Part model, mm, in its own coordinate system. A direction names the side the tool comes from. Give positions to 0.01 mm unless a question says otherwise; leave off trailing zeros. Loops run counter-clockwise (first coordinate to the right, second up) from the corner with the lowest first, then second, coordinate; pieces in that order, holes last. Notation, with made-up numbers: (35, -22) -> (80, -22) arc R23 cw to (80, 9) -> close; hole circle Ø9 at (37.25, 32). An arc over 180 degrees is marked (long way). One line per question, with ' | ' between items.
```python
from build123d import *

# Parameters (mm, degrees)
BOSS_EXTRUDE1_DEPTH          = 65
CUT_EXTRUDE1_DEPTH           = 92.186621826
CUT_EXTRUDE1_DEPTH_BACK      = 92.186621826
SKETCH3_R                    = 9
CUT_EXTRUDE2_DEPTH           = 8
CUT_EXTRUDE3_START           = -8
SKETCH4_R                    = 9
CUT_EXTRUDE3_DEPTH           = 8
M16_TAPPED_HOLE1_D           = 14
M16_TAPPED_HOLE1_CSINK_D     = 16.05
M16_TAPPED_HOLE1_CSINK_ANGLE = 90
M12_TAPPED_HOLE1_D           = 10.2
M12_TAPPED_HOLE1_CSINK_D     = 12.05
M12_TAPPED_HOLE1_CSINK_ANGLE = 90


with BuildPart() as part:
    # Sketch1 → Boss-Extrude1 (new body)
    with BuildSketch(Plane.XY):
        Polygon((16.5, 0), (-16.5, 0), (-17, 0.5), (-17, 13.5), (-16.5, 14), (-12.707106781, 14), (-12, 13.292893219), (-11.292893219, 14), (-12, 14.707106781), (-12, 56.5), (-11.5, 57), (11.5, 57), (12, 56.5), (12, 14.707106781), (11.292893219, 14), (12, 13.292893219), (12.707106781, 14), (16.5, 14), (17, 13.5), (17, 0.5), align=None)
    extrude(amount=BOSS_EXTRUDE1_DEPTH)

    # Sketch2 → Cut-Extrude1 (cut, two sides: drawn at the far end of the back side and taken through both)
    with BuildSketch(Plane(origin=(12, 0, 0), x_dir=(0, 0, -1), z_dir=(1, 0, 0)).offset(-CUT_EXTRUDE1_DEPTH_BACK)):
        Polygon((-40, 79.715196203), (7.535961079, 79.715196203), (7.535961079, 25), (-39.292893219, 25), (-40, 24.292893219), (-40.707106781, 25), (-40, 25.707106781), align=None)
    extrude(amount=CUT_EXTRUDE1_DEPTH + CUT_EXTRUDE1_DEPTH_BACK, mode=Mode.SUBTRACT)

    # Sketch3 → Cut-Extrude2 (cut)
    with BuildSketch(Plane.XY.offset(65)):
        with Locations((0, 12)):
            Circle(SKETCH3_R)
    extrude(amount=-CUT_EXTRUDE2_DEPTH, mode=Mode.SUBTRACT)

    # Sketch4 → Cut-Extrude3 (cut)
    with BuildSketch(Plane(origin=(0, 0, 0), x_dir=(-1, 0, 0), z_dir=(0, 0, -1)).offset(CUT_EXTRUDE3_START)):
        with Locations(Location((0, 12, 0), (0, 0, 180))):
            Circle(SKETCH4_R)
    extrude(amount=CUT_EXTRUDE3_DEPTH, mode=Mode.SUBTRACT)

    # M16 Tapped Hole1 (through all)
    with Locations(Plane(origin=(0, 12, 8), x_dir=(-1, 0, 0), z_dir=(0, 0, -1))):
        with Locations((0, 0)):
            CounterSinkHole(M16_TAPPED_HOLE1_D / 2, M16_TAPPED_HOLE1_CSINK_D / 2, counter_sink_angle=M16_TAPPED_HOLE1_CSINK_ANGLE)

    # M12 Tapped Hole1 (through all)
    with Locations(Plane(origin=(0, 42, 65), x_dir=(1, 0, 0), z_dir=(0, 0, 1))):
        with Locations((0, 0)):
            CounterSinkHole(M12_TAPPED_HOLE1_D / 2, M12_TAPPED_HOLE1_CSINK_D / 2, counter_sink_angle=M12_TAPPED_HOLE1_CSINK_ANGLE)


solid = part.part
```
1) Saw through at D-D (z = 29.5). Give the cut face in (x, y), and give its area (3 significant figures).
Found:
outline: (-17, 0.5) -> (-16.5, 0) -> (16.5, 0) -> (17, 0.5) -> (17, 13.5) -> (16.5, 14) -> (12.71, 14) -> (12, 13.29) -> (11.29, 14) -> (12, 14.71) -> (12, 25) -> (-12, 25) -> (-12, 14.71) -> (-11.29, 14) -> (-12, 13.29) -> (-12.71, 14) -> (-16.5, 14) -> (-17, 13.5) -> close; hole circle Ø14 at (0, 12) | area: 584 mm2
2) Tool access for faces 5 (the flat face through (0, 4.7, 57)), 6 (the cylindrical face through (-1.951, 20.786, 4.056)), 7 (the flat face through (-6, 41, 40)), 8 (the flat face through (15, 14, 32)): list every direction of +Z, -Z, +X, -X, +Y, -Y with a clear straight run to the whole face (end or side of a thin tool).
Found:
face 5: +Z | face 6: -Z | face 7: -Z, +X, -X, +Y | face 8: +Z, -Z, +X, +Y
3) Saw through at C-C (z = 46). Give the cut face in (x, y), and give its area (3 significant figures).
Found:
outline: (-17, 0.5) -> (-16.5, 0) -> (16.5, 0) -> (17, 0.5) -> (17, 13.5) -> (16.5, 14) -> (12.71, 14) -> (12, 13.29) -> (11.29, 14) -> (12, 14.71) -> (12, 56.5) -> (11.5, 57) -> (-11.5, 57) -> (-12, 56.5) -> (-12, 14.71) -> (-11.29, 14) -> (-12, 13.29) -> (-12.71, 14) -> (-16.5, 14) -> (-17, 13.5) -> close; hole circle Ø14 at (0, 12); hole circle Ø10.2 at (0, 42) | area: 1,270 mm2
4) Saw through at B-B (x = 0). State how many separate pieces and enclosed holes the cut face has, and give its area (3 significant figures).
Found:
separate pieces: 3 | enclosed holes: 0 | area: 1,190 mm2
5) Pull direction X, two halves, no side cores. Call faces 1 (the cylindrical face through (-1.517, 5.166, 33.348)), 2 (the flat face through (-12, 31, 46)), 3 (the cylindrical face through (-1.951, 3.214, 61.056)), 4 (the flat face through (0, 25, 19)): pulls with the +X half, pulls with the -X half, needs draft (parallel to the pull), parting line crosses it, or undercut.
Found:
face 1: undercut | face 2: pulls with the -X half | face 3: undercut | face 4: needs draft
6) Drill centre lines: line 1 (Y direction, x = 0, z = 59); line 2 (Y direction, x = 0, z = 33); line 3 (Y direction, x = 0, z = 43). Where is each one in solid material? Low to high.
Found:
line 1: 0 to 3, 21 to 36.9, 47.1 to 57 | line 2: 0 to 5, 19 to 25 | line 3: 0 to 5, 19 to 36.9, 47.1 to 57
7) Saw through at A-A (y = 42). Give the cut face in (x, z) (3 decimals), and give its area (3 significant figures).
Found:
outline: (-12, 40) -> (-5.1, 40) -> (-5.1, 64.075) -> (-6.025, 65) -> (-12, 65) -> close; (5.1, 40) -> (12, 40) -> (12, 65) -> (6.025, 65) -> (5.1, 64.075) -> close | area: 344 mm2
8) Pin check, flat tips, straight feed: P1, Ø1.9, axis at x = -14.5, z = 42.5, coming from the +Y side; P2, Ø10, axis at x = -2, y = 43, coming from the -Z side; P3, Ø6, axis at x = -6.5, z = 18, coming from the -Y side; P4, Ø16, axis at x = 0, y = 12, coming from the -Z side (3 decimals). Stop position of each tip, or through.
Found:
P1: y = 14 | P2: z = 40 | P3: y = 0 | P4: z = 8.025
